from build123d import *

# Parameters (mm, degrees)
BOSS_EXTRUDE1_DEPTH = 3
CHAMFER1_SIZE       = 35


with BuildPart() as part:
    # Sketch1 → Boss-Extrude1 (new, symmetric)
    with BuildSketch(Plane.XY):
        Polygon((0, 100), (0, 0), (75, 0), (75, 10), (10, 100), align=None)
    extrude(amount=BOSS_EXTRUDE1_DEPTH, both=True)

    # Chamfer1
    chamfer1_edges = [part.edges().sort_by_distance(p)[0] for p in [
        (0, 0, 0),
    ]]
    chamfer(chamfer1_edges, length=CHAMFER1_SIZE)


solid = part.part
The model under review builds one solid part; all positions refer to its coordinate system, in mm. Round coordinates to 2 decimals unless told otherwise and drop trailing zeros. Write each loop counter-clockwise with the first axis right and the second up, starting at its lowest first coordinate (ties: lowest second). Pieces come first, ordered by that corner, then holes. Notation, with made-up numbers: M 18,23 L 27,23 A15 cw 27,37 Z; hole C 39,75.25 d8. An arc over 180 degrees is marked long. Use a Markdown table: item, result. Add a question column.
Q1. We need section B-B, the plane y = 43. State the section outline as (x, z) points.
Q2. Insertion check: pin 1 (8 mm diameter, centred on x = 15.5, y = 10.5, fed in from +Z); pin 2 (1 mm diameter, centred on x = 29.5, z = 0.5, fed in from -Y); pin 3 (1.5 mm diameter, centred on y = 64, z = 0.5, fed in from +X); pin 4 (1.5 mm diameter, centred on x = 33.5, z = 2, fed in from -Y). Each pin has a flat end and moves straight along its axis. Give the tip position at first contact, or say it passes through.
Q3. We need section A-A, the plane x = 5. State the section outline as (y, z) points, plus the area to 3 significant figures.
Q4. To check wall thickness, follow line 1 (Y direction, x = 44, z = -2); line 2 (Y direction, x = 15.5, z = -1.5); line 3 (X direction, y = 83, z = 1). State the ranges of each line that lie inside material, in increasing order.
Findings below:
| question | item | result |
|---|---|---|
| 1 | outline | M 0,-3 L 51.17,-3 L 51.17,3 L 0,3 Z |
| 2 | pin 1 | passes through |
| 2 | pin 2 | stops at y = 5 |
| 2 | pin 3 | stops at x = 36.54 |
| 2 | pin 4 | stops at y = 0.75 |
| 3 | outline | M 30,-3 L 100,-3 L 100,3 L 30,3 Z |
| 3 | area | 420 mm² |
| 4 | line 1 | y = 0 to 52.92 |
| 4 | line 2 | y = 19.5 to 92.38 |
| 4 | line 3 | x = 0 to 22.28 |
